from build123d import *

# Parameters (mm, degrees)
SKETCH_2_R          = 60
EXTRUDE_1_DEPTH     = 80
SKETCH_1_R          = 37.5
CUT_EXTRUDE_1_DEPTH = 60
CUT_EXTRUDE_START   = -20
CUT_EXTRUDE_2_DEPTH = 20
SKETCH_4_W          = 20
SKETCH_4_H          = 11.668393693
CUT_EXTRUDE_3_DEPTH = 30


with BuildPart() as part:
    # 草图2 → 凸台-拉伸1 (new body)
    with BuildSketch(Plane.XY):
        Circle(SKETCH_2_R)
    extrude(amount=EXTRUDE_1_DEPTH)

    # 草图1 → 切除-拉伸1 (cut)
    with BuildSketch(Plane.XY):
        Circle(SKETCH_1_R)
    extrude(amount=CUT_EXTRUDE_1_DEPTH, mode=Mode.SUBTRACT)

    # 草图3 → 切除-拉伸2 (cut)
    with BuildSketch(Plane.XY.offset(80).offset(CUT_EXTRUDE_START)):
        with BuildLine():
            Line((57.811529494, 16.05699404), (46.47114317, 9.509618943))
            Line((46.47114317, 9.509618943), (31.47114317, 35.490381057))
            Line((31.47114317, 35.490381057), (42.811529494, 42.037756153))
            ThreePointArc((42.811529494, 42.037756153), (51.961524227, 30), (57.811529494, 16.05699404))
        make_face()
        with BuildLine():
            Line((-15, 58.094750193), (-15, 45))
            Line((-15, 45), (15, 45))
            Line((15, 45), (15, 58.094750193))
            ThreePointArc((15, 58.094750193), (0, 60), (-15, 58.094750193))
        make_face()
        with BuildLine():
            Line((42.811529494, -42.037756153), (31.47114317, -35.490381057))
            Line((31.47114317, -35.490381057), (46.47114317, -9.509618943))
            Line((46.47114317, -9.509618943), (57.811529494, -16.05699404))
            ThreePointArc((57.811529494, -16.05699404), (51.961524227, -30), (42.811529494, -42.037756153))
        make_face()
        with BuildLine():
            Line((-15, -58.094750193), (-15, -45))
            Line((-15, -45), (15, -45))
            Line((15, -45), (15, -58.094750193))
            ThreePointArc((15, -58.094750193), (0, -60), (-15, -58.094750193))
        make_face()
        with BuildLine():
            Line((-57.811529494, -16.05699404), (-46.47114317, -9.509618943))
            Line((-46.47114317, -9.509618943), (-31.47114317, -35.490381057))
            Line((-31.47114317, -35.490381057), (-42.811529494, -42.037756153))
            ThreePointArc((-42.811529494, -42.037756153), (-51.961524227, -30), (-57.811529494, -16.05699404))
        make_face()
        with BuildLine():
            Line((-42.811529494, 42.037756153), (-31.47114317, 35.490381057))
            Line((-31.47114317, 35.490381057), (-46.47114317, 9.509618943))
            Line((-46.47114317, 9.509618943), (-57.811529494, 16.05699404))
            ThreePointArc((-57.811529494, 16.05699404), (-51.961524227, 30), (-42.811529494, 42.037756153))
        make_face()
    extrude(amount=CUT_EXTRUDE_2_DEPTH, mode=Mode.SUBTRACT)

    # 草图4 → 切除-拉伸3 (cut)
    with BuildSketch(Plane(origin=(0, 0, 0), x_dir=(-1, 0, 0), z_dir=(0, 0, -1))):
        with Locations((0, 34.165803154)):
            Rectangle(SKETCH_4_W, SKETCH_4_H)
    extrude(amount=-CUT_EXTRUDE_3_DEPTH, mode=Mode.SUBTRACT)


solid = part.part
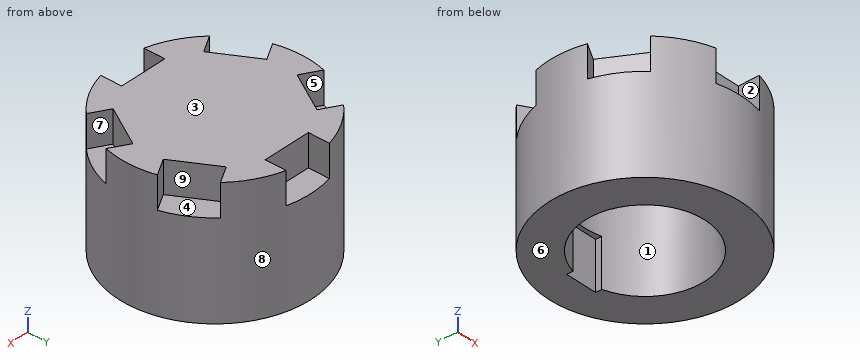
The model under review builds one solid part; all positions refer to its coordinate system, in mm. Face numbers are marked on the shaded views. A direction names the side the tool comes from. Give positions to 0.01 mm unless a question says otherwise; leave off trailing zeros. Loops run counter-clockwise (first coordinate to the right, second up) from the corner with the lowest first, then second, coordinate; pieces in that order, holes last. Notation, with made-up numbers: (69.25, -8) -> (127.25, -8) arc R23 ccw to (127.25, 31) -> close; hole circle Ø6 at (19, 82.25). An arc over 180 degrees is marked (long way). Put each result on its own line as item: value. Start each with the question number.
1. Clearance check with flat-ended pins moving along their axes: P1, Ø2, axis at x = 28, y = 16, coming from the -Z side; P2, Ø1.9, axis at y = 38.5, z = 17, coming from the +X side; P3, Ø3, axis at y = 47, z = 32.5, coming from the -X side; P4, Ø8, axis at x = 39, y = 22.5, coming from the +Z side. State where each tip first meets the part, or that it passes through.
2. Mouldability with a two-part tool opening along X and no side actions: class the marked faces 6, 7, 8 and 9 as released by +X, released by -X, zero draft, split by the parting line, or undercut.
3. We need section B-B on y = 0. State the section outline as (x, z) points.
4. We need section D-D on z = 74.5. State the section outline as (x, y) points, then the cut area to 3 significant figures.
5. For the marked faces 1, 2, 3, 4 and 5, list the 3-axis set-ups (+Z, -Z, +X, -X, +Y, -Y) from which the entire face can be reached by the end or side of a thin tool; tool diameter is ignored.
6. Wall thickness on probe 1 along Y at (x, z) = (0, 23.5); probe 2 along Y at (x, z) = (0, 31.5): over which ranges is each line inside the solid? List them lowest first.
7. We need section C-C on x = 0. State the section outline as (y, z) points.
8. We need section A-A on z = 10. State the section outline as (x, y) points, then the cut area to 3 significant figures.
Determined:
1. P1: z = 60
1. P2: x = 46.8
1. P3: x = -39.11
1. P4: z = 80
2. face 6: zero draft
2. face 7: released by +X
2. face 8: split by the parting line
2. face 9: undercut
3. outline: (-60, 0) -> (-37.5, 0) -> (-37.5, 60) -> (37.5, 60) -> (37.5, 0) -> (60, 0) -> (60, 80) -> (-60, 80) -> close
4. outline: (-57.81, -16.06) -> (-46.47, -9.51) -> (-31.47, -35.49) -> (-42.81, -42.04) arc R60 ccw to (-15, -58.09) -> (-15, -45) -> (15, -45) -> (15, -58.09) arc R60 ccw to (42.81, -42.04) -> (31.47, -35.49) -> (46.47, -9.51) -> (57.81, -16.06) arc R60 ccw to (57.81, 16.06) -> (46.47, 9.51) -> (31.47, 35.49) -> (42.81, 42.04) arc R60 ccw to (15, 58.09) -> (15, 45) -> (-15, 45) -> (-15, 58.09) arc R60 ccw to (-42.81, 42.04) -> (-31.47, 35.49) -> (-46.47, 9.51) -> (-57.81, 16.06) arc R60 ccw to start
4. area: 8,720 mm^2
5. face 1: -Z
5. face 2: +Z, -Y
5. face 3: +Z, +X, -X, +Y, -Y
5. face 4: +Z
5. face 5: +Z, +Y
6. probe 1: -60 to -37.5, 40 to 60
6. probe 2: -60 to -37.5, 37.5 to 60
7. outline: (-60, 0) -> (-37.5, 0) -> (-37.5, 60) -> (37.5, 60) -> (37.5, 30) -> (40, 30) -> (40, 0) -> (60, 0) -> (60, 60) -> (45, 60) -> (45, 80) -> (-45, 80) -> (-45, 60) -> (-60, 60) -> close
8. outline: circle Ø120 at (0, 0); hole (-10, 36.14) arc R37.5 ccw (long way) to (10, 36.14) -> (10, 40) -> (-10, 40) -> close
8. area: 6,830 mm^2
